from build123d import *

# Parameters (mm, degrees)
SKETCH1_W           = 400
SKETCH1_H           = 400
SKETCH1_R           = 16
BOSS_EXTRUDE1_DEPTH = 10


with BuildPart() as part:
    # Sketch1 → Boss-Extrude1 (new body)
    with BuildSketch(Plane.XY):
        Rectangle(SKETCH1_W, SKETCH1_H)
        with Locations((-160, 160)):
            Circle(SKETCH1_R, mode=Mode.SUBTRACT)
        with Locations((160, 160)):
            Circle(SKETCH1_R, mode=Mode.SUBTRACT)
        with Locations((160, -160)):
            Circle(SKETCH1_R, mode=Mode.SUBTRACT)
        with Locations((-160, -160)):
            Circle(SKETCH1_R, mode=Mode.SUBTRACT)
    extrude(amount=BOSS_EXTRUDE1_DEPTH)


solid = part.part
Source: CAD feature listing. Evaluate the final solid. Frame: model axes, mm. Give positions to 0.01 mm unless a question says otherwise; leave off trailing zeros. Write each loop counter-clockwise with the first axis right and the second up, starting at its lowest first coordinate (ties: lowest second). Pieces come first, ordered by that corner, then holes. Notation, with made-up numbers: M -16.75,2.5 L 13.25,2.5 A8 cw 13.25,9.5 Z; hole C 49,-38 d6. An arc over 180 degrees is marked long. Return JSON: item names as keys, results as strings. Group by question number.
1) Cut plane A-A, the plane y = -160. Output: boundary loops of the cut face in (x, z), plus the area to 3 significant figures.
2) Material intervals for line 1 along Y through (x, z) = (160, 3.75); line 2 along X through (y, z) = (-164.5, 3); line 3 along X through (y, z) = (-171.5, 8), sorted ascending. Write a range as [from, to].
3) Pull-direction query (X, two-part tool) for faces 1 (the face through (-162.083, -144.136, 4.93)), 2 (the face through (-3, 3, 0)), 3 (the face through (200, -3, 5)); classes: pulls with the +X half, pulls with the -X half, needs draft (parallel to the pull), parting line crosses it, or undercut.
4) Cut plane C-C, the plane z = 3.25. Output: boundary loops of the cut face in (x, y), plus the area to 3 significant figures.
Recorded:
{
 "1": {"outline": "M -200,0 L -176,0 L -176,10 L -200,10 Z; M -144,0 L 144,0 L 144,10 L -144,10 Z; M 176,0 L 200,0 L 200,10 L 176,10 Z", "area": "3,360 mm²"},
 "2": {"line 1": "y = [-200, -176], [-144, 144], [176, 200]", "line 2": "x = [-200, -175.35], [-144.65, 144.65], [175.35, 200]", "line 3": "x = [-200, -171.12], [-148.88, 148.88], [171.12, 200]"},
 "3": {"face 1": "undercut", "face 2": "needs draft", "face 3": "pulls with the +X half"},
 "4": {"outline": "M -200,-200 L 200,-200 L 200,200 L -200,200 Z; hole C -160,-160 d32; hole C -160,160 d32; hole C 160,-160 d32; hole C 160,160 d32", "area": "157,000 mm²"}
}
